```python
from build123d import *

# Parameters (mm, degrees)
SKETCH_2_R          = 11
SKETCH_2_R_2        = 13.5
SKETCH_2_R_3        = 2.25
EXTRUDE_1_DEPTH     = 10
CHAMFER_1_SIZE      = 20
CUT_EXTRUDE_1_REACH = 192.164
SKETCH_3_R          = 2.5


with BuildPart() as part:
    # 草图2 → 凸台-拉伸1 (new body)
    with BuildSketch(Plane.XY):
        Polygon((-22.5, 67.5), (177.5, 67.5), (177.5, 12.5), (22.5, 12.5), (22.5, -22.5), (-22.5, -22.5), align=None)
        Circle(SKETCH_2_R, mode=Mode.SUBTRACT)
        with Locations((0, 45)):
            Circle(SKETCH_2_R_2, mode=Mode.SUBTRACT)
        with Locations((-16.5, 61.5)):
            Circle(SKETCH_2_R_3, mode=Mode.SUBTRACT)
        with Locations(Location((16.5, 61.5, 0), (0, 0, 180))):
            Circle(SKETCH_2_R_3, mode=Mode.SUBTRACT)
        with Locations((16.5, 28.5)):
            Circle(SKETCH_2_R_3, mode=Mode.SUBTRACT)
        with Locations(Location((-16.5, 28.5, 0), (0, 0, 180))):
            Circle(SKETCH_2_R_3, mode=Mode.SUBTRACT)
        with Locations((0, 16)):
            Circle(SKETCH_2_R_3, mode=Mode.SUBTRACT)
        with Locations((16, 0)):
            Circle(SKETCH_2_R_3, mode=Mode.SUBTRACT)
        with Locations((0, -16)):
            Circle(SKETCH_2_R_3, mode=Mode.SUBTRACT)
        with Locations((-16, 0)):
            Circle(SKETCH_2_R_3, mode=Mode.SUBTRACT)
        with BuildLine():
            Line((162, 47), (82, 47))
            ThreePointArc((82, 47), (76.5, 52.5), (82, 58))
            Line((82, 58), (162, 58))
            ThreePointArc((162, 58), (167.5, 52.5), (162, 47))
        make_face(mode=Mode.SUBTRACT)
        with BuildLine():
            Line((162, 33), (82, 33))
            ThreePointArc((82, 33), (76.5, 27.5), (82, 22))
            Line((82, 22), (162, 22))
            ThreePointArc((162, 22), (167.5, 27.5), (162, 33))
        make_face(mode=Mode.SUBTRACT)
    extrude(amount=EXTRUDE_1_DEPTH)

    # 倒角1
    chamfer_1_edges = [part.edges().sort_by_distance(p)[0] for p in [
        (22.5, 12.5, 5),
    ]]
    chamfer(chamfer_1_edges, length=CHAMFER_1_SIZE)

    # 草图3 → 切除-拉伸1 (cut, up to next)
    with BuildSketch(Plane(origin=(0, 0, 0), x_dir=(-1, 0, 0), z_dir=(0, 0, -1)), mode=Mode.PRIVATE) as cut_extrude_1_sk1:
        with Locations((-57, 55.5)):
            Circle(SKETCH_3_R)
    cut_extrude_1_tool1 = extrude(cut_extrude_1_sk1.sketch, amount=-CUT_EXTRUDE_1_REACH, mode=Mode.PRIVATE) & part.part
    # 草图3 → 切除-拉伸1 (cut, up to next)
    with BuildSketch(Plane(origin=(0, 0, 0), x_dir=(-1, 0, 0), z_dir=(0, 0, -1)), mode=Mode.PRIVATE) as cut_extrude_1_sk2:
        with Locations((-33, 55.5)):
            Circle(SKETCH_3_R)
    cut_extrude_1_tool2 = extrude(cut_extrude_1_sk2.sketch, amount=-CUT_EXTRUDE_1_REACH, mode=Mode.PRIVATE) & part.part
    # 草图3 → 切除-拉伸1 (cut, up to next)
    with BuildSketch(Plane(origin=(0, 0, 0), x_dir=(-1, 0, 0), z_dir=(0, 0, -1)), mode=Mode.PRIVATE) as cut_extrude_1_sk3:
        with Locations((-33, 31.5)):
            Circle(SKETCH_3_R)
    cut_extrude_1_tool3 = extrude(cut_extrude_1_sk3.sketch, amount=-CUT_EXTRUDE_1_REACH, mode=Mode.PRIVATE) & part.part
    # 草图3 → 切除-拉伸1 (cut, up to next)
    with BuildSketch(Plane(origin=(0, 0, 0), x_dir=(-1, 0, 0), z_dir=(0, 0, -1)), mode=Mode.PRIVATE) as cut_extrude_1_sk4:
        with Locations((-57, 31.5)):
            Circle(SKETCH_3_R)
    cut_extrude_1_tool4 = extrude(cut_extrude_1_sk4.sketch, amount=-CUT_EXTRUDE_1_REACH, mode=Mode.PRIVATE) & part.part
    add(cut_extrude_1_tool1.solids().sort_by_distance((57, 55.5, 0))[0], mode=Mode.SUBTRACT)
    add(cut_extrude_1_tool2.solids().sort_by_distance((33, 55.5, 0))[0], mode=Mode.SUBTRACT)
    add(cut_extrude_1_tool3.solids().sort_by_distance((33, 31.5, 0))[0], mode=Mode.SUBTRACT)
    add(cut_extrude_1_tool4.solids().sort_by_distance((57, 31.5, 0))[0], mode=Mode.SUBTRACT)


solid = part.part
```
The listing builds one solid part. Answer for the finished solid, in the listing's coordinates (mm). A direction names the side the tool comes from. Coordinates: 2 decimals unless noted, no trailing zeros. Order: outer loops, then holes, each group sorted by start corner. A loop starts at its lowest first (then second) coordinate and runs counter-clockwise, first axis right, second up. Notation, with made-up numbers: M -1.5,28 L 7.5,28 A14 ccw 7.5,35 Z; hole C -37,52.25 d3. An arc over 180 degrees is marked long. Answer as a JSON object with one key per item and string values. Group by question number.
1. Straight lines are drawn through the part: line 1 (Y direction, x = 57, z = 7); line 2 (Y direction, x = 126, z = 5.25); line 3 (Y direction, x = 0, z = 8). For each, find the intervals that lie inside material, in ascending order.
2. Section B-B on y = -16 is taken. Write down the section's boundary in (x, z).
3. Flat-ended cylindrical pins translate along their axes: P1, Ø3, axis at x = 118, z = 4.5, coming from the -Y side; P2, Ø1, axis at x = 40, z = 2, coming from the -Y side; P3, Ø6, axis at y = 0, z = 2.5, coming from the +X side. Find the tip coordinate at first contact, or state that the pin passes through.
4. Section C-C on z = 6.75 is taken. State how many separate pieces and enclosed holes the cut face has, then the cut area to 3 significant figures.
5. Section D-D on y = 61.5 is taken. Write down the section's boundary in (x, z), then the cut area to 3 significant figures.
6. A tool of negligible diameter and unlimited length cuts with its end or side. For faces 4 (the flat face through (79, 33, 0)), 5 (the flat face through (123, 33, 5)), from which of +Z, -Z, +X, -X, +Y, -Y can it reach the whole face along a straight path? Write none if from no direction.
7. Determine the mould class of faces 1 (the cylindrical face through (54.69, 54.54, 4.93)), 2 (the flat face through (22.5, -15, 5)), 3 (the flat face through (111, 12.5, 5)) for opening direction X: released by +X, released by -X, zero draft, split by the parting line, or undercut.
8. Section A-A on x = 0 is taken. Write down the section's boundary in (y, z), then the cut area to 3 significant figures.
Values follow:
{
 "1": {"line 1": "12.5 to 29, 34 to 53, 58 to 67.5", "line 2": "12.5 to 22, 33 to 47, 58 to 67.5", "line 3": "-22.5 to -18.25, -13.75 to -11, 11 to 13.75, 18.25 to 31.5, 58.5 to 67.5"},
 "2": {"outline": "M -22.5,0 L -2.25,0 L -2.25,10 L -22.5,10 Z; M 2.25,0 L 22.5,0 L 22.5,10 L 2.25,10 Z"},
 "3": {"P1": "y = 12.5", "P2": "y = 9.5", "P3": "x = 33"},
 "4": {"separate pieces": "1", "enclosed holes": "16", "area": "9,670 mm2"},
 "5": {"outline": "M -22.5,0 L -18.75,0 L -18.75,10 L -22.5,10 Z; M -14.25,0 L 14.25,0 L 14.25,10 L -14.25,10 Z; M 18.75,0 L 177.5,0 L 177.5,10 L 18.75,10 Z", "area": "1,910 mm2"},
 "6": {"face 4": "-Z, +X, -X, +Y, -Y", "face 5": "+Z, -Z"},
 "7": {"face 1": "undercut", "face 2": "released by +X", "face 3": "zero draft"},
 "8": {"outline": "M -22.5,0 L -18.25,0 L -18.25,10 L -22.5,10 Z; M -13.75,0 L -11,0 L -11,10 L -13.75,10 Z; M 11,0 L 13.75,0 L 13.75,10 L 11,10 Z; M 18.25,0 L 31.5,0 L 31.5,10 L 18.25,10 Z; M 58.5,0 L 67.5,0 L 67.5,10 L 58.5,10 Z", "area": "320 mm2"}
}
